from build123d import *

# Parameters (mm, degrees)
GB_T_6728_2002_RECTANGULAR_HOLLOW_SECTIO_DEPTH = 884
F_13_0_13_DIAMETER_HOLE1_D                     = 13


with BuildPart() as part:
    # Sketch14 → GB/T 6728-2002 rectangular hollow section 60X40X5(1) (new body)
    with BuildSketch(Plane(origin=(0, 0, 0), x_dir=(-1, 0, 0), z_dir=(0, 1, 0))):
        with BuildLine():
            Line((-12, -30), (12, -30))
            ThreePointArc((12, -30), (17.656854249, -27.656854249), (20, -22))
            Line((20, -22), (20, 22))
            ThreePointArc((20, 22), (17.656854249, 27.656854249), (12, 30))
            Line((12, 30), (-12, 30))
            ThreePointArc((-12, 30), (-17.656854249, 27.656854249), (-20, 22))
            Line((-20, 22), (-20, -22))
            ThreePointArc((-20, -22), (-17.656854249, -27.656854249), (-12, -30))
        make_face()
        with BuildLine():
            Line((-12, -25), (12, -25))
            ThreePointArc((12, -25), (14.121320344, -24.121320344), (15, -22))
            Line((15, -22), (15, 22))
            ThreePointArc((15, 22), (14.121320344, 24.121320344), (12, 25))
            Line((12, 25), (-12, 25))
            ThreePointArc((-12, 25), (-14.121320344, 24.121320344), (-15, 22))
            Line((-15, 22), (-15, -22))
            ThreePointArc((-15, -22), (-14.121320344, -24.121320344), (-12, -25))
        make_face(mode=Mode.SUBTRACT)
    extrude(amount=GB_T_6728_2002_RECTANGULAR_HOLLOW_SECTIO_DEPTH)

    # Ø13.0 (13) Diameter Hole1 (through all)
    with Locations(Plane.XY.offset(30)):
        with Locations((0, 414), (0, 314)):
            Hole(F_13_0_13_DIAMETER_HOLE1_D / 2)


solid = part.part
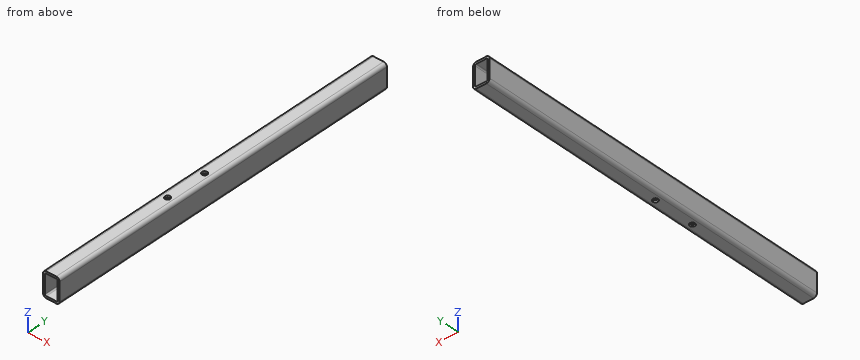
Build history of the part. All positions in model axes, mm. Round coordinates to 2 decimals unless told otherwise and drop trailing zeros. Loops run counter-clockwise (first coordinate to the right, second up) from the corner with the lowest first, then second, coordinate; pieces in that order, holes last. Notation, with made-up numbers: (70, 23) -> (123, 23) arc R24 ccw to (123, 50) -> close; hole circle Ø11 at (-16, 40.5). An arc over 180 degrees is marked (long way). Answer in a Markdown table with one row per item.
Item 1: Saw through at B-B (x = 0). Write the cut outline in (y, z).
Answers below:
| item | result |
|---|---|
| outline | (0, -30) -> (307.5, -30) -> (307.5, -25) -> (0, -25) -> close; (0, 25) -> (307.5, 25) -> (307.5, 30) -> (0, 30) -> close; (320.5, -30) -> (407.5, -30) -> (407.5, -25) -> (320.5, -25) -> close; (320.5, 25) -> (407.5, 25) -> (407.5, 30) -> (320.5, 30) -> close; (420.5, -30) -> (884, -30) -> (884, -25) -> (420.5, -25) -> close; (420.5, 25) -> (884, 25) -> (884, 30) -> (420.5, 30) -> close |
Item 2: Pin check, flat tips, straight feed: pin 1 (12 mm diameter, centred on x = -7.5, z = -16, fed in from -Y); pin 2 (2 mm diameter, centred on y = 509.5, z = 24, fed in from +X). Stop position of each tip, or through.
Answers below:
| item | result |
|---|---|
| pin 1 | passes through |
| pin 2 | stops at x = 19.94 |
Item 3: Saw through at C-C (y = 602.5). Write the cut outline in (x, z).
Answers below:
| item | result |
|---|---|
| outline | (-20, -22) arc R8 ccw to (-12, -30) -> (12, -30) arc R8 ccw to (20, -22) -> (20, 22) arc R8 ccw to (12, 30) -> (-12, 30) arc R8 ccw to (-20, 22) -> close; hole (-15, -22) arc R3 ccw to (-12, -25) -> (12, -25) arc R3 ccw to (15, -22) -> (15, 22) arc R3 ccw to (12, 25) -> (-12, 25) arc R3 ccw to (-15, 22) -> close |
Item 4: Saw through at A-A (z = -3.5). Write the cut outline in (x, y), and give its area (3 significant figures).
Answers below:
| item | result |
|---|---|
| outline | (-20, 0) -> (-15, 0) -> (-15, 884) -> (-20, 884) -> close; (15, 0) -> (20, 0) -> (20, 884) -> (15, 884) -> close |
| area | 8,840 mm² |
Item 5: Drill centre lines: L1, parallel to Y at x = 0, z = 26.35; L2, parallel to Z at x = -8, y = 193.5; L3, parallel to X at y = 519, z = 9. Where is each one in solid material? Low to high. Write a range as [from, to].
Answers below:
| item | result |
|---|---|
| L1 | y = [0, 307.5], [320.5, 407.5], [420.5, 884] |
| L2 | z = [-30, -25], [25, 30] |
| L3 | x = [-20, -15], [15, 20] |
